```python
from build123d import *

# Parameters (mm, degrees)
BOSS_EXTRUDE1_DEPTH = 10
CUT_EXTRUDE8_DEPTH  = 10
SKETCH21_R          = 6
CUT_EXTRUDE14_DEPTH = 36
CUT_EXTRUDE15_DEPTH = 10
SKETCH19_R          = 125.517206862
CUT_EXTRUDE16_DEPTH = 10


with BuildPart() as part:
    # Sketch1 → Boss-Extrude1 (new body)
    with BuildSketch(Plane.XY):
        Polygon((0, 0), (0, 170), (100, 170), (100, 0), (100, -20), (0, -20), align=None)
    extrude(amount=BOSS_EXTRUDE1_DEPTH)

    # Sketch9 → Cut-Extrude8 (cut)
    with BuildSketch(Plane.XY.offset(10)):
        with BuildLine():
            Line((29.787758795, 148.908841534), (29.787758795, 138.908841534))
            ThreePointArc((29.787758795, 138.908841534), (35.787758795, 132.908841534), (41.787758795, 138.908841534))
            Line((41.787758795, 138.908841534), (41.787758795, 148.908841534))
            ThreePointArc((41.787758795, 148.908841534), (35.787758795, 154.908841534), (29.787758795, 148.908841534))
        make_face()
    extrude(amount=-CUT_EXTRUDE8_DEPTH, mode=Mode.SUBTRACT)

    # Sketch21 → Cut-Extrude14 (cut)
    with BuildSketch(Plane(origin=(0, 0, 0), x_dir=(-1, 0, 0), z_dir=(0, 0, -1))):
        with Locations((-51.483180233, 14.944928588)):
            Circle(SKETCH21_R)
        with Locations((-173.125589471, 5.899139524)):
            Circle(SKETCH21_R)
    extrude(amount=-CUT_EXTRUDE14_DEPTH, mode=Mode.SUBTRACT)

    # Sketch28 → Cut-Extrude15 (cut)
    with BuildSketch(Plane.XY.offset(10)):
        with BuildLine():
            ThreePointArc((78.796565751, 119.119536449), (75.600421883, 126.979858603), (67.740099728, 123.783714736))
            add(Edge.make_bspline(
                [(67.740099728, 123.783714736), (64.092305086, 115.480107597), (59.109492341, 103.369529902), (53.161827647, 83.940069885), (51.100576539, 72.87588046), (49.983799811, 65.743090583)],
                knots=[0, 0, 0, 0, 0.446952238, 0.644100667, 1, 1, 1, 1], degree=3))
            ThreePointArc((49.983799811, 65.743090583), (55.659355828, 58.49601037), (62.288867459, 64.882064178))
            add(Edge.make_bspline(
                [(78.796565751, 119.119536449), (75.230202559, 110.937069208), (70.252785241, 99.033521906), (65.59137225, 83.75023837), (63.459360665, 73.923916137), (62.602399905, 67.882836475), (62.288867459, 64.882064178)],
                knots=[0, 0, 0, 0, 0.457699653, 0.660132463, 0.817976892, 0.972547387, 0.972547387, 0.972547387, 0.972547387], degree=3))
        make_face()
    extrude(amount=-CUT_EXTRUDE15_DEPTH, mode=Mode.SUBTRACT)

    # Sketch19 → Cut-Extrude16 (cut)
    # profile 1 of 2: a face of its own
    with BuildSketch(Plane.XY.offset(10)):
        with Locations((58.773015823, 71.241859079)):
            Circle(SKETCH19_R)
        with BuildLine():
            Line((41.881776011, 59.878203095), (36.689834848, 17.426245238))
            ThreePointArc((36.689834848, 17.426245238), (49.776196121, 0.042371585), (66.454445821, 14.016916355))
            Line((66.454445821, 14.016916355), (70.10422157, 59.327257721))
            Line((70.10422157, 59.327257721), (70.725023214, 61.382630275))
            Line((70.725023214, 61.382630275), (87.508098537, 116.948643541))
            ThreePointArc((87.508098537, 116.948643541), (87.335113551, 126.939388183), (80.925197211, 134.604756721))
            Line((80.925197211, 134.604756721), (43.432736819, 156.814433772))
            ThreePointArc((43.432736819, 156.814433772), (26.883190667, 155.979826019), (21.200543901, 140.414108121))
            Line((21.200543901, 140.414108121), (41.325983429, 62.042545062))
            Line((41.325983429, 62.042545062), (41.881776011, 59.878203095))
        make_face(mode=Mode.SUBTRACT)
    # profile 2 of 2: a face of its own
    with BuildSketch(Plane.XY.offset(10)):
        with BuildLine():
            Line((52.121181326, 136.108026927), (36.779697673, 111.015745375))
            ThreePointArc((36.779697673, 111.015745375), (36.33960448, 109.402281892), (36.831704565, 107.803912744))
            Line((36.831704565, 107.803912744), (41.662593186, 100.448764157))
            ThreePointArc((41.662593186, 100.448764157), (44.33499195, 99.10023877), (46.84322719, 100.733943719))
            Line((46.84322719, 100.733943719), (62.827881658, 132.111730058))
            ThreePointArc((62.827881658, 132.111730058), (62.851731636, 134.787382647), (60.730080577, 136.417806633))
            Line((60.730080577, 136.417806633), (55.25602114, 137.487450431))
            ThreePointArc((55.25602114, 137.487450431), (53.472410109, 137.289048664), (52.121181326, 136.108026927))
        make_face()
    extrude(amount=-CUT_EXTRUDE16_DEPTH, mode=Mode.SUBTRACT)


solid = part.part
```
Can you work these out from the model? Positions are in its coordinate system, mm. A direction names the side the tool comes from. Give positions to 0.01 mm unless a question says otherwise; leave off trailing zeros. Order: outer loops, then holes, each group sorted by start corner. A loop starts at its lowest first (then second) coordinate and runs counter-clockwise, first axis right, second up. Notation, with made-up numbers: M 59,52.25 L 83,52.25 A24 cw 83,82.25 Z; hole C 64.25,88 d7. An arc over 180 degrees is marked long. Write item = value, one per line. Start each with the question number.
Q1. Suppose I cut it at B-B (y = 45.5). Write out the boundary of the cut face in (x, z).
Q2. Suppose I cut it at D-D (y = 23). Write out the boundary of the cut face in (x, z).
Q3. I need wall thicknesses on probe 1 along X at (y, z) = (124, 4.25); probe 2 along X at (y, z) = (105, 2.75); probe 3 along Y at (x, z) = (49.5, 9.25). Which ranges of each line are inside material? Lowest first, please. Write a range as [from, to].
Q4. Suppose I cut it at A-A (x = 33). Write out the boundary of the cut face in (y, z), plus the area to 3 significant figures.
Q5. Will these pins go through, and if not, where does the flat tip stop? pin 1 Ø10 at (x, y) = (68.5, 45) entering from -Z; pin 2 Ø2 at (y, z) = (124, 2.5) entering from +X.
Q6. We'd pull the mould along X, two halves only. Please class faces 4 (the cylindrical face through (49.438, 0.085, 5.07)), 5 (the cylindrical face through (75.72, 126.93, 5.07)), 6 (the cylindrical face through (87.384, 126.806, 5.07)): pulls with the +X half, pulls with the -X half, needs draft (parallel to the pull), parting line crosses it, or undercut.
Q7. Suppose I cut it at C-C (z = 5.5). Count the separate pieces of the cut face and the enclosed holes in it, plus the area to 3 significant figures.
Q8. For faces 1 (the flat face through (39.322, 38.949, 5.07)), 2 (the flat face through (29.788, 144, 5)), 3 (the flat face through (68.254, 36.355, 5.07)), which set-ups out of +Z, -Z, +X, -X, +Y, -Y let a thin tool reach every point of the face, with its end or its side?
Check result:
q1.outline = M 40.12,0 L 68.99,0 L 68.99,10 L 40.12,10 Z
q2.outline = M 37.37,0 L 67.18,0 L 67.18,10 L 37.37,10 Z
q3.probe_1 = [25.42, 44.72], [58.7, 67.84], [78.7, 88.1]
q3.probe_2 = [30.29, 38.67], [49.02, 60.05], [72.88, 83.9]
q3.probe_3 = [0.08, 9.28], [20.61, 105.95], [131.82, 153.22]
q4.outline = M 94.47,0 L 133.6,0 L 133.6,10 L 94.47,10 Z; M 154.22,0 L 158.65,0 L 158.65,10 L 154.22,10 Z
q4.area = 436 mm2
q5.pin_1 = 0
q5.pin_2 = 88.22
q6.face_4 = parting line crosses it
q6.face_5 = undercut
q6.face_6 = pulls with the +X half
q7.separate_pieces = 1
q7.enclosed_holes = 4
q7.area = 4,540 mm2
q8.face_1 = +Z, -Z, -X
q8.face_2 = +Z, -Z
q8.face_3 = +Z, -Z, +X, -Y
